CAD build for the part. Positions are in the model's coordinates, mm. A direction names the side the tool comes from. Round coordinates to 2 decimals unless told otherwise and drop trailing zeros. Order: outer loops, then holes, each group sorted by start corner. A loop starts at its lowest first (then second) coordinate and runs counter-clockwise, first axis right, second up. Notation, with made-up numbers: (-23.5, 35) - (32.5, 35) arc R17 ccw to (32.5, 44) - close; hole circle Ø9 at (38.25, 8). An arc over 180 degrees is marked (long way). Use one line per item in the form item = value. Start each with the question number.
from build123d import *

# Parameters (mm, degrees)
SADDLE_BODY_DEPTH                      = 25
CORNER_POCKET_34X22_DEPTH              = 15
CORNER_POCKET_MIRROR_SIDE_COPY_1_DEPTH = 15
BORE_SKETCH_R                          = 15
BORE_30_DEPTH                          = 83.637763765
BORE_PLUG_SKETCH_R                     = 15
BORE_PLUG_DEPTH                        = 15
PLUG_SLOT_SKETCH_W                     = 10
PLUG_SLOT_SKETCH_H                     = 8
PLUG_SLOT_8X10_DEPTH                   = 15


with BuildPart() as part:
    # Saddle Profile Sketch → Saddle Body (new, symmetric)
    with BuildSketch(Plane.XY):
        Polygon((-45, 0), (-45, 10), (-30, 48), (30, 48), (45, 10), (45, 0), (26, 0), (26, -12), (-26, -12), (-26, 0), align=None)
    extrude(amount=SADDLE_BODY_DEPTH, both=True)

    # Corner Pocket Sketch → Corner Pocket 34x22 (cut)
    with BuildSketch(Plane.XY.offset(25)):
        Polygon((-30, 48), (-22, 48), (-22, 22), (-40.263157895, 22), align=None)
    corner_pocket_34x22 = extrude(amount=-CORNER_POCKET_34X22_DEPTH, mode=Mode.SUBTRACT)

    # Corner Pocket Mirror Front: Corner Pocket 34x22 across plane
    add(corner_pocket_34x22.mirror(Plane.XY), mode=Mode.SUBTRACT)

    # Corner Pocket Mirror Side: Corner Pocket 34x22 across plane
    add(corner_pocket_34x22.mirror(Plane(origin=(0, 0, 0), x_dir=(0, 0, 1), z_dir=(1, 0, 0))), mode=Mode.SUBTRACT)

    # Corner Pocket Mirror Side copy 1 sketch → Corner Pocket Mirror Side copy 1 (cut)
    with BuildSketch(Plane(origin=(0, 0, -25), x_dir=(-1, 0, 0), z_dir=(0, 0, -1))):
        Polygon((-30, 48), (-22, 48), (-22, 22), (-40.263157895, 22), align=None)
    extrude(amount=-CORNER_POCKET_MIRROR_SIDE_COPY_1_DEPTH, mode=Mode.SUBTRACT)

    # Bore Sketch → Bore Ø30 (cut, through all)
    with BuildSketch(Plane.XY.offset(25)):
        with Locations((0, 48)):
            Circle(BORE_SKETCH_R)
    extrude(amount=-BORE_30_DEPTH, mode=Mode.SUBTRACT)

    # Bore Plug Sketch → Bore Plug (add, symmetric)
    with BuildSketch(Plane.XY):
        with Locations((0, 48)):
            Circle(BORE_PLUG_SKETCH_R)
    extrude(amount=BORE_PLUG_DEPTH, both=True)

    # Plug Slot Sketch → Plug Slot 8x10 (cut, symmetric)
    with BuildSketch(Plane(origin=(0, 0, 0), x_dir=(0, 0, -1), z_dir=(1, 0, 0))):
        with Locations((10, 59)):
            Rectangle(PLUG_SLOT_SKETCH_W, PLUG_SLOT_SKETCH_H)
    plug_slot_8x10 = extrude(amount=PLUG_SLOT_8X10_DEPTH, both=True, mode=Mode.SUBTRACT)

    # Plug Slot Mirror: Plug Slot 8x10 across plane
    add(plug_slot_8x10.mirror(Plane.XY), mode=Mode.SUBTRACT)


solid = part.part
(1) Slice it at A-A (z = -7.5). Give the cut face in (x, y), and give its area (3 significant figures).
(2) Mould opens along X. For faces 4 (the flat face through (-29, 32, -10)), 5 (the cylindrical face through (0, 33, 20)), 6 (the flat face through (-22, 35, -18)) say: pulls with the +X half, pulls with the -X half, needs draft (parallel to the pull), parting line crosses it, or undercut.
(3) Flat gauge pins, fed straight in: P1, Ø2, axis at y = 28, z = 0.5, coming from the +X side; P2, Ø2.5, axis at x = -3, y = 59, coming from the +Z side; P3, Ø12, axis at x = -33, z = -16.5, coming from the +Y side. Where does each tip first touch, or does it go through?
(4) Slice it at D-D (z = -20.5). Give the cut face in (x, y), and give its area (3 significant figures).
(5) Wall check: line 1 (Y direction, x = 38.5, z = 12); line 2 (Y direction, x = 22, z = -1); line 3 (X direction, y = 26.5, z = -23). Give the ranges that are in metal, low to high. Write a range as [from, to].
(6) Slice it at C-C (y = 38). Give the cut face in (x, z).
(7) Slice it at B-B (x = 0). Give the cut face in (y, z).
(8) Which spindle directions (+Z, -Z, +X, -X, +Y, -Y) get a long thin tool onto all of the face, cutting with end or side? Do faces 1 (the flat face through (0, 58, -5)), 2 (the flat face through (31, 22, 18)), 3 (the flat face through (-31, 22, 18)). Say none if no direction does.
Results list:
q1.outline = (-45, 0) - (-26, 0) - (-26, -12) - (26, -12) - (26, 0) - (45, 0) - (45, 10) - (30, 48) - (15, 48) arc R15 ccw to (13.27, 55) - (-13.27, 55) arc R15 ccw to (-15, 48) - (-30, 48) - (-45, 10) - close
q1.area = 4,580 mm²
q2.face_4 = needs draft
q2.face_5 = undercut
q2.face_6 = pulls with the -X half
q3.P1 = 38.29
q3.P2 = 5
q3.P3 = 22
q4.outline = (-45, 0) - (-26, 0) - (-26, -12) - (26, -12) - (26, 0) - (45, 0) - (45, 10) - (40.26, 22) - (22, 22) - (22, 48) - (15, 48) arc R15 cw to (-15, 48) - (-22, 48) - (-22, 22) - (-40.26, 22) - (-45, 10) - close
q4.area = 3,340 mm²
q5.line_1 = [0, 22]
q5.line_2 = [-12, 48]
q5.line_3 = [-22, 22]
q6.outline = (-33.95, -10) - (-22, -10) - (-22, -25) - (-11.18, -25) - (-11.18, -15) - (11.18, -15) - (11.18, -25) - (22, -25) - (22, -10) - (33.95, -10) - (33.95, 10) - (22, 10) - (22, 25) - (11.18, 25) - (11.18, 15) - (-11.18, 15) - (-11.18, 25) - (-22, 25) - (-22, 10) - (-33.95, 10) - close
q7.outline = (-12, -25) - (33, -25) - (33, -15) - (55, -15) - (55, -5) - (63, -5) - (63, 5) - (55, 5) - (55, 15) - (33, 15) - (33, 25) - (-12, 25) - close
q8.face_1 = -Z, +X, -X, +Y
q8.face_2 = +Z, +X, +Y
q8.face_3 = +Z, -X, +Y
